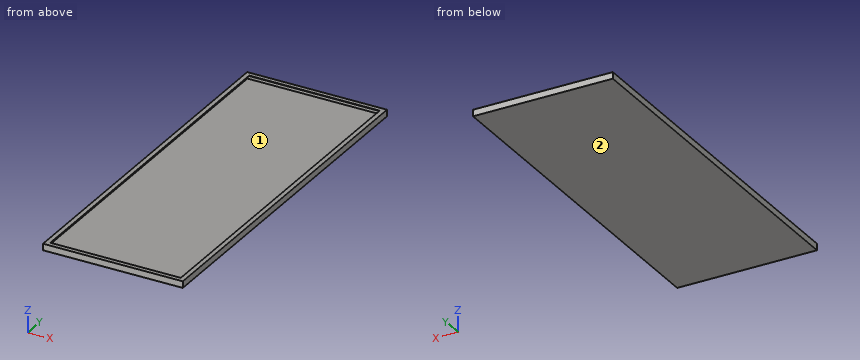
```python
from build123d import *

# Parameters (mm, degrees)
SKETCH_1_W      = 601
SKETCH_1_H      = 1551
EXTRUDE_1_DEPTH = 28
SHELL_1_T       = -2
SKETCH_2_W      = 601
SKETCH_2_H      = 1551
SKETCH_2_W_2    = 561
SKETCH_2_H_2    = 1511
EXTRUDE_2_DEPTH = 2


with BuildPart() as part:
    # 草图1 → 凸台-拉伸1 (new body)
    with BuildSketch(Plane.XY):
        with Locations((300.5, 775.5)):
            Rectangle(SKETCH_1_W, SKETCH_1_H)
    extrude(amount=EXTRUDE_1_DEPTH)

    # 抽壳1
    shell_1_openings = [part.faces().sort_by_distance(p)[0] for p in [
        (300.5, 775.5, 28),
    ]]
    offset(amount=SHELL_1_T, openings=shell_1_openings, kind=Kind.INTERSECTION)

    # 草图2 → 凸台-拉伸2 (add)
    with BuildSketch(Plane.XY.offset(28)):
        with Locations((300.5, 775.5)):
            Rectangle(SKETCH_2_W, SKETCH_2_H)
        with Locations((300.5, 775.5)):
            Rectangle(SKETCH_2_W_2, SKETCH_2_H_2, mode=Mode.SUBTRACT)
    extrude(amount=-EXTRUDE_2_DEPTH)


solid = part.part
```
Geometry check sheet. Reference: the model listing, model coordinates, mm. Face numbers are marked on the shaded views. Coordinates: 2 decimals unless noted, no trailing zeros. Loops run counter-clockwise (first coordinate to the right, second up) from the corner with the lowest first, then second, coordinate; pieces in that order, holes last.
Item 1: Thickness scan on line 1 (X direction, y = 993.5, z = 19); line 2 (Y direction, x = 514, z = 8); line 3 (Y direction, x = 95, z = 26.5). Record the ranges inside material, lowest first.
Item 2: Sectioned sample at A-A, the plane z = 13.75. Record the boundary of the cut face in (x, y).
Item 3: Release check for a two-part mould opening along Y. For the marked faces 1 and 2 record: released by +Y, released by -Y, zero draft, split by the parting line, or undercut.
Item 4: Sectioned sample at C-C, the plane y = 409. Record the boundary of the cut face in (x, z), then the cut area to 3 significant figures.
Item 5: Sectioned sample at B-B, the plane x = 313. Record the boundary of the cut face in (y, z).
Check result:
1. line 1: x = 0 to 2, 599 to 601
1. line 2: y = 0 to 2, 1549 to 1551
1. line 3: y = 0 to 20, 1531 to 1551
2. outline: (0, 0) - (601, 0) - (601, 1551) - (0, 1551) - close; hole (2, 2) - (599, 2) - (599, 1549) - (2, 1549) - close
3. face 1: undercut
3. face 2: zero draft
4. outline: (0, 0) - (601, 0) - (601, 28) - (581, 28) - (581, 26) - (599, 26) - (599, 2) - (2, 2) - (2, 26) - (20, 26) - (20, 28) - (0, 28) - close
4. area: 1,380 mm2
5. outline: (0, 0) - (1551, 0) - (1551, 28) - (1531, 28) - (1531, 26) - (1549, 26) - (1549, 2) - (2, 2) - (2, 26) - (20, 26) - (20, 28) - (0, 28) - close
